Geometry check sheet. Reference: drawing and pictorial views, mm from the part's lowest x, y, z. A direction names the side the tool comes from. Round coordinates to 2 decimals unless told otherwise and drop trailing zeros. Write each loop counter-clockwise with the first axis right and the second up, starting at its lowest first coordinate (ties: lowest second). Pieces come first, ordered by that corner, then holes. Notation, with made-up numbers: (-34, 14) -> (0, 14) arc R25 ccw to (0, 38) -> close; hole circle Ø8 at (50, 16). An arc over 180 degrees is marked (long way). Write item = value, one per line.
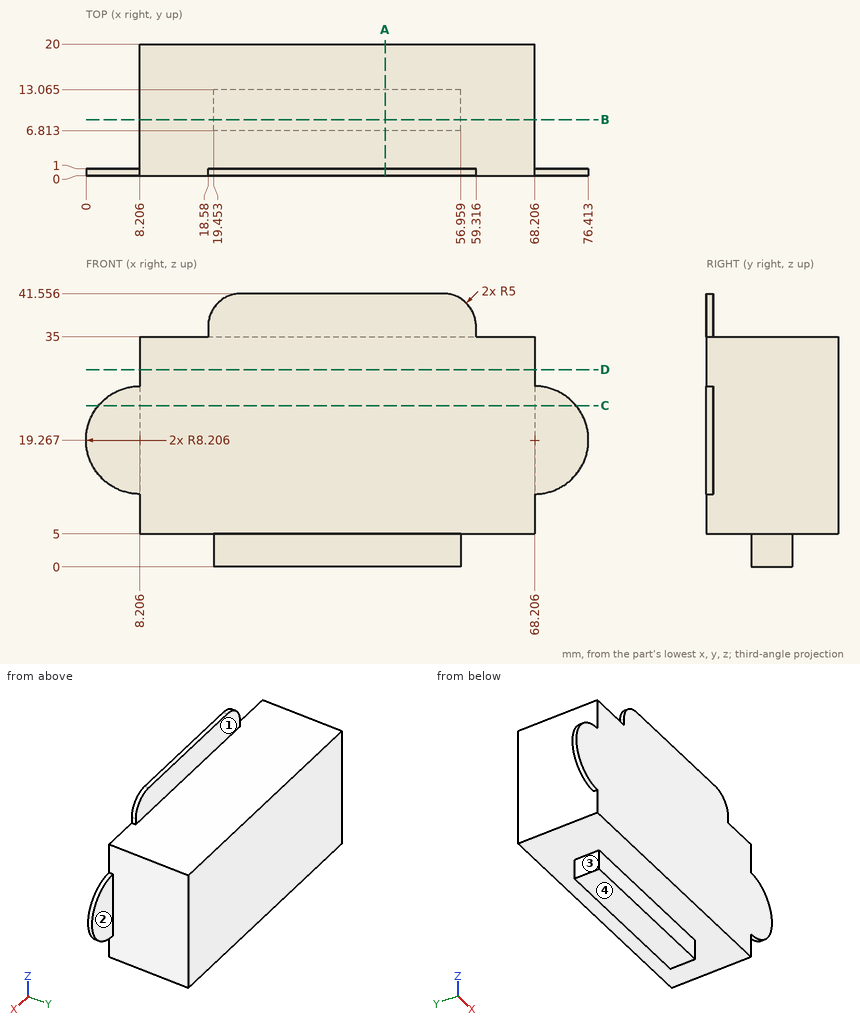
(1) Sectioned sample at B-B on y = 8.5. Enter the section's corners in (x, z), then the cut area to 3 significant figures.
Worked answers:
outline = (8.21, 5) -> (19.45, 5) -> (19.45, 0) -> (56.96, 0) -> (56.96, 5) -> (68.21, 5) -> (68.21, 35) -> (8.21, 35) -> close
area = 1,990 mm²
(2) Go/stop test with flat-tipped pins: P1, Ø5.5, axis at y = 8.5, z = 3, coming from the -X side; P2, Ø10, axis at y = 13, z = 17.5, coming from the +X side; P3, Ø1.5, axis at x = 30.5, z = 2.5, coming from the -Y side. Record where each tip stops, or that it passes through.
Worked answers:
P1 = 8.21
P2 = 68.21
P3 = 6.81
(3) Sectioned sample at D-D on z = 30. Enter the section's corners in (x, y), then the cut area to 3 significant figures.
Worked answers:
outline = (8.21, 0) -> (68.21, 0) -> (68.21, 20) -> (8.21, 20) -> close
area = 1,200 mm²
(4) Access from +Z, -Z, +X, -X, +Y, -Y to the whole of each face (thin tool, end or side, straight path). Record for the marked faces 1, 2, 3 and 4.
Worked answers:
face_1 = +Z, +X, -X, +Y
face_2 = +Z, -Z, +X, +Y
face_3 = -Z, -X, +Y, -Y
face_4 = -Z, +X, -X, +Y, -Y
(5) Sectioned sample at C-C on z = 24.5. Enter the section's corners in (x, y) (1 decimal).
Worked answers:
outline = (1.9, 0) -> (74.5, 0) -> (74.5, 1) -> (68.2, 1) -> (68.2, 20) -> (8.2, 20) -> (8.2, 1) -> (1.9, 1) -> close
(6) Sectioned sample at A-A on x = 45.5. Enter the section's corners in (y, z) (1 decimal), then the cut area to 3 significant figures.
Worked answers:
outline = (0, 5) -> (6.8, 5) -> (6.8, 0) -> (13.1, 0) -> (13.1, 5) -> (20, 5) -> (20, 35) -> (1, 35) -> (1, 41.6) -> (0, 41.6) -> close
area = 638 mm²
(7) Material ranges on L1, parallel to X at y = 11.5, z = 2; L2, parallel to Y at x = 26, z = 36; L3, parallel to Z at x = 49.5, y = 8.25, recorded low to high. Write a range as [from, to].
Worked answers:
L1 = [19.45, 56.96]
L2 = [0, 1]
L3 = [0, 35]
